from build123d import *

# Parameters (mm, degrees)
BASE_DEPTH = 695
FILLET1_R  = 8.5
FILLET2_R  = 4.25


with BuildPart() as part:
    # Sketch1 → Base (new body)
    with BuildSketch(Plane(origin=(0, 0, -28.211262136), x_dir=(0, 0, 1), z_dir=(1, 0, 0))):
        Polygon((28.211262136, -50), (28.211262136, 50), (76.211262136, 50), (76.211262136, 43.635), (33.511262136, 39.365), (33.511262136, -39.365), (76.211262136, -43.635), (76.211262136, -50), align=None)
    extrude(amount=BASE_DEPTH)

    # Fillet1
    fillet1_edges = [part.edges().sort_by_distance(p)[0] for p in [
        (347.5, -39.365, 5.3),
        (347.5, 39.365, 5.3),
    ]]
    fillet(fillet1_edges, radius=FILLET1_R)

    # Fillet2
    fillet2_edges = [part.edges().sort_by_distance(p)[0] for p in [
        (347.5, 43.635, 48),
        (347.5, -43.635, 48),
    ]]
    fillet(fillet2_edges, radius=FILLET2_R)


solid = part.part
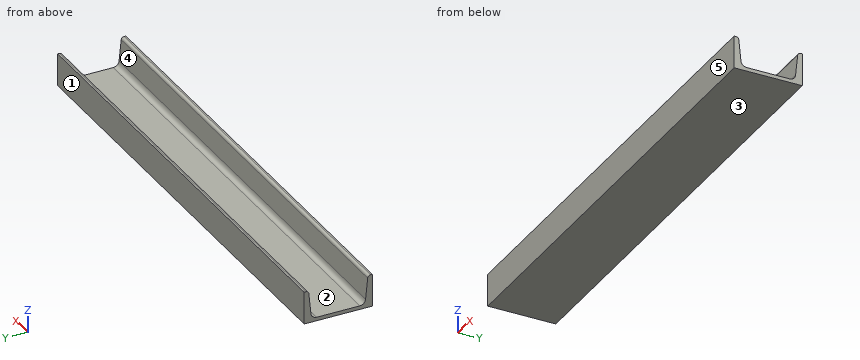
Build history of the part. All positions in model axes, mm. Face numbers are marked on the shaded views. A direction names the side the tool comes from. Round coordinates to 2 decimals unless told otherwise and drop trailing zeros. Loops run counter-clockwise (first coordinate to the right, second up) from the corner with the lowest first, then second, coordinate; pieces in that order, holes last. Notation, with made-up numbers: (50, -11) -> (108, -11) arc R34 cw to (108, 28) -> close; hole circle Ø9 at (83, 38). An arc over 180 degrees is marked (long way). Use CSV: the item, a comma, the result in double quotes. Start each with the question number.
Q1. Saw through at C-C on y = 13. Give the cut face in (x, z), and give its area (3 significant figures).
Q2. Saw through at A-A on z = 30.5. Give the cut face in (x, y) (3 decimals), and give its area (3 significant figures).
Q3. Drill centre lines: L1, parallel to Y at x = 584, z = 43 (3 decimals); L2, parallel to Z at x = 622, y = 33; L3, parallel to Z at x = 155.5, y = 45.5. Where is each one in solid material? Low to high.
Q4. Which spindle directions (+Z, -Z, +X, -X, +Y, -Y) get a long thin tool onto all of the face, cutting with end or side? Do the marked faces 1 and 2. Say none if no direction does.
Q5. Saw through at B-B on x = 219.5. Give the cut face in (y, z), and give its area (3 significant figures).
Q6. Mould opens along Y. For the marked faces 3, 4 and 5 say: +Y half, -Y half, draft (parallel to the pull), parting line (faces both ways), or undercut.
Solutions:
1,outline,"(0, 0) -> (695, 0) -> (695, 5.3) -> (0, 5.3) -> close"
1,area,"3,680 mm^2"
2,outline,"(0, -50) -> (695, -50) -> (695, -41.885) -> (0, -41.885) -> close; (0, 41.885) -> (695, 41.885) -> (695, 50) -> (0, 50) -> close"
2,area,"11,300 mm^2"
3,L1,"y = -50 to -43.135, 43.135 to 50"
3,L2,"z = 0 to 5.4"
3,L3,"z = 0 to 47.51"
4,face 1,"+Z, -Z, +X, -X, +Y"
4,face 2,"+Z, +X, -X"
5,outline,"(-50, 0) -> (50, 0) -> (50, 48) -> (47.48, 48) arc R4.25 ccw to (43.25, 44.17) -> (40.13, 12.95) arc R8.5 cw to (31.67, 5.3) -> (-31.67, 5.3) arc R8.5 cw to (-40.13, 12.95) -> (-43.25, 44.17) arc R4.25 ccw to (-47.48, 48) -> (-50, 48) -> close"
5,area,"1,270 mm^2"
6,face 3,"draft"
6,face 4,"undercut"
6,face 5,"-Y half"
